For this review, take the finished solid that the model builds, in its own axes (mm). Give positions to 0.01 mm unless a question says otherwise; leave off trailing zeros. Loops run counter-clockwise (first coordinate to the right, second up) from the corner with the lowest first, then second, coordinate; pieces in that order, holes last. Notation, with made-up numbers: (83.5, 14) -> (132.5, 14) arc R36 cw to (132.5, 49) -> close; hole circle Ø2 at (19.5, -17). An arc over 180 degrees is marked (long way). Answer as CSV lines item,"result". Start each with the question number.
Item 1: Add section A-A on z = -13. State the section outline as (x, y) points, plus the area to 3 significant figures.
Item 2: Add section C-C on x = 37. State the section outline as (y, z) points, plus the area to 3 significant figures.
Item 3: For L1, parallel to X at y = 3.8, z = -13; L2, parallel to X at y = 1.65, z = -15; L3, parallel to Z at x = -38, y = 0.65, list the stretches that pass through material, from the lowest coordinate up. Write a range as from..to.
Item 4: Add section B-B on y = 1.5. State the section outline as (x, z) points, plus the area to 3 significant figures.
Item 5: The part is to be moulded in two halves that separate along Z. For faces 1 (the face through (45, 2, 0)), 2 (the face through (39.727, 2.535, -13.358)), 3 (the face through (-1, 2, 30)), say which applies: +Z half, -Z half, draft (parallel to the pull), parting line (faces both ways), or undercut.
```python
from build123d import *

# Parameters (mm, degrees)
SKETCH_1_W          = 90
SKETCH_1_H          = 60
EXTRUDE_1_DEPTH     = 5
CHAMFER_1_SIZE      = 3
SKETCH_2_R          = 2.75
CUT_EXTRUDE_1_DEPTH = 10


with BuildPart() as part:
    # 草图1 → 凸台-拉伸1 (new body)
    with BuildSketch(Plane(origin=(0, 0, 0), x_dir=(1, 0, 0), z_dir=(0, 1, 0))):
        Rectangle(SKETCH_1_W, SKETCH_1_H)
    extrude(amount=EXTRUDE_1_DEPTH)

    # 倒角1
    chamfer_1_edges = [part.edges().sort_by_distance(p)[0] for p in [
        (45, 2.5, 30),
        (-45, 2.5, 30),
        (-45, 2.5, -30),
        (45, 2.5, -30),
    ]]
    chamfer(chamfer_1_edges, length=CHAMFER_1_SIZE)

    # 草图2 → 切除-拉伸1 (cut)
    with BuildSketch(Plane(origin=(0, 5, 0), x_dir=(1, 0, 0), z_dir=(0, 1, 0))):
        with Locations(Location((37, -17, 0), (0, 0, 270))):
            Circle(SKETCH_2_R)
        with Locations(Location((-37, -17, 0), (0, 0, 270))):
            Circle(SKETCH_2_R)
        with Locations(Location((37, 13, 0), (0, 0, 270))):
            Circle(SKETCH_2_R)
        with Locations(Location((-37, 13, 0), (0, 0, 270))):
            Circle(SKETCH_2_R)
    extrude(amount=-CUT_EXTRUDE_1_DEPTH, mode=Mode.SUBTRACT)


solid = part.part
```
Computed values:
1,outline,"(-45, 0) -> (-39.75, 0) -> (-39.75, 5) -> (-45, 5) -> close; (-34.25, 0) -> (34.25, 0) -> (34.25, 5) -> (-34.25, 5) -> close; (39.75, 0) -> (45, 0) -> (45, 5) -> (39.75, 5) -> close"
1,area,"395 mm²"
2,outline,"(0, -30) -> (5, -30) -> (5, -15.75) -> (0, -15.75) -> close; (0, -10.25) -> (5, -10.25) -> (5, 14.25) -> (0, 14.25) -> close; (0, 19.75) -> (5, 19.75) -> (5, 30) -> (0, 30) -> close"
2,area,"245 mm²"
3,L1,"-45..-39.75, -34.25..34.25, 39.75..45"
3,L2,"-45..-38.89, -35.11..35.11, 38.89..45"
3,L3,"-30..-15.56, -10.44..14.44, 19.56..30"
4,outline,"(-45, -27) -> (-42, -30) -> (42, -30) -> (45, -27) -> (45, 27) -> (42, 30) -> (-42, 30) -> (-45, 27) -> close; hole circle Ø5.5 at (-37, -13); hole circle Ø5.5 at (-37, 17); hole circle Ø5.5 at (37, -13); hole circle Ø5.5 at (37, 17)"
4,area,"5,290 mm²"
5,face 1,"draft"
5,face 2,"undercut"
5,face 3,"+Z half"
